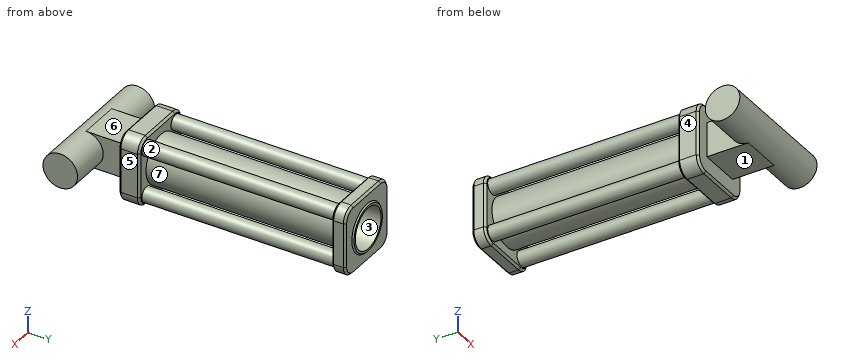
```python
from build123d import *

# Parameters (mm, degrees)
SKETCH1_R                = 175
SKETCH1_R_2              = 150
BOSS_EXTRUDE1_DEPTH      = 1500
SKETCH2_W                = 500
SKETCH2_H                = 500
BOSS_EXTRUDE2_DEPTH      = 150
BOSS_EXTRUDE3_DEPTH      = 150
BOSS_EXTRUDE3_DEPTH_BACK = 150
BOSS_EXTRUDE4_DEPTH      = 450
BOSS_EXTRUDE4_DEPTH_BACK = 450
SKETCH4_R                = 125
CHAMFER2_SIZE            = 10
SKETCH5_W                = 500
SKETCH5_H                = 500
SKETCH5_R                = 154.887495166
BOSS_EXTRUDE5_DEPTH      = 100
BOSS_EXTRUDE6_REACH      = 1587.875
SKETCH6_R                = 54.226637303
CIRPATTERN1_COUNT        = 4
FILLET1_R                = 90
CHAMFER3_SIZE            = 15


with BuildPart() as part:
    # Sketch1 → Boss-Extrude1 (new body)
    with BuildSketch(Plane(origin=(0, 0, 0), x_dir=(1, 0, 0), z_dir=(0, 1, 0))):
        with Locations(Location((0, 0, 0), (0, 0, 270))):
            Circle(SKETCH1_R)
        with Locations(Location((0, 0, 0), (0, 0, 270))):
            Circle(SKETCH1_R_2, mode=Mode.SUBTRACT)
    extrude(amount=BOSS_EXTRUDE1_DEPTH)

    # Sketch2 → Boss-Extrude2 (add)
    with BuildSketch(Plane.XZ):
        Rectangle(SKETCH2_W, SKETCH2_H)
    extrude(amount=BOSS_EXTRUDE2_DEPTH)

    # Sketch3 → Boss-Extrude3 (add, two sides: drawn at the far end of the back side and taken through both)
    with BuildSketch(Plane(origin=(0, 0, 0), x_dir=(0, 0, -1), z_dir=(1, 0, 0)).offset(-BOSS_EXTRUDE3_DEPTH_BACK)):
        with BuildLine():
            Line((125, -150), (125, -450))
            ThreePointArc((125, -450), (0, -575), (-125, -450))
            Line((-125, -450), (-125, -150))
            Line((-125, -150), (125, -150))
        make_face()
    extrude(amount=BOSS_EXTRUDE3_DEPTH + BOSS_EXTRUDE3_DEPTH_BACK)

    # Sketch4 → Boss-Extrude4 (add, two sides: drawn at the far end of the back side and taken through both)
    with BuildSketch(Plane(origin=(0, 0, 0), x_dir=(0, 0, -1), z_dir=(1, 0, 0)).offset(-BOSS_EXTRUDE4_DEPTH_BACK)):
        with Locations((0, -450)):
            Circle(SKETCH4_R)
    extrude(amount=BOSS_EXTRUDE4_DEPTH + BOSS_EXTRUDE4_DEPTH_BACK)

    # Chamfer2
    chamfer2_edges = [part.edges().sort_by_distance(p)[0] for p in [
        (0, 1500, -175),
    ]]
    chamfer(chamfer2_edges, length=CHAMFER2_SIZE)

    # Sketch5 → Boss-Extrude5 (add)
    with BuildSketch(Plane(origin=(0, 1490, 0), x_dir=(1, 0, 0), z_dir=(0, 1, 0))):
        Rectangle(SKETCH5_W, SKETCH5_H)
        Circle(SKETCH5_R, mode=Mode.SUBTRACT)
    extrude(amount=-BOSS_EXTRUDE5_DEPTH)

    # Sketch6 → Boss-Extrude6 (add, up to next)
    with BuildSketch(Plane(origin=(0, 0, 0), x_dir=(1, 0, 0), z_dir=(0, 1, 0)), mode=Mode.PRIVATE) as boss_extrude6_sk1:
        with Locations(Location((-170.275340777, 170.275340777, 0), (0, 0, 90))):
            Circle(SKETCH6_R)
    boss_extrude6_tool1 = extrude(boss_extrude6_sk1.sketch, amount=BOSS_EXTRUDE6_REACH, mode=Mode.PRIVATE) - part.part
    boss_extrude6 = boss_extrude6_tool1.solids().sort_by_distance((-170.275341, 0, -170.275341))[0]
    add(boss_extrude6)

    # CirPattern1: Boss-Extrude6 ×4 about axis
    cirpattern1_axis = Axis((0, 0, 0), (0, 1, 0))
    for i in range(1, CIRPATTERN1_COUNT):
        add(boss_extrude6.rotate(cirpattern1_axis, i * 360 / CIRPATTERN1_COUNT))

    # Fillet1
    fillet1_edges = [part.edges().sort_by_distance(p)[0] for p in [
        (250, -75, -250),
        (250, -75, 250),
        (-250, -75, 250),
        (-250, -75, -250),
        (250, 1440, -250),
        (250, 1440, 250),
        (-250, 1440, 250),
        (-250, 1440, -250),
    ]]
    fillet(fillet1_edges, radius=FILLET1_R)

    # Chamfer3
    chamfer3_edges = [part.edges().sort_by_distance(p)[0] for p in [
        (250, -150, 0),
        (0, 0, -250),
        (-250, 0, 0),
        (0, 0, 250),
        (-223.639610307, 0, -223.639610307),
        (-223.639610307, 0, 223.639610307),
        (223.639610307, 0, 223.639610307),
        (223.639610307, 0, -223.639610307),
        (0, -150, -250),
        (0, -150, 250),
        (-250, -150, 0),
        (-223.639610307, -150, -223.639610307),
        (-223.639610307, -150, 223.639610307),
        (223.639610307, -150, 223.639610307),
        (223.639610307, -150, -223.639610307),
        (0, 1490, -250),
        (0, 1390, -250),
        (250, 1490, 0),
        (-250, 1490, 0),
        (0, 1490, 250),
        (223.639610307, 1490, -223.639610307),
        (223.639610307, 1490, 223.639610307),
        (-223.639610307, 1490, 223.639610307),
        (-223.639610307, 1490, -223.639610307),
        (-250, 1390, 0),
        (250, 1390, 0),
        (0, 1390, 250),
        (223.639610307, 1390, -223.639610307),
        (223.639610307, 1390, 223.639610307),
        (-223.639610307, 1390, 223.639610307),
        (-223.639610307, 1390, -223.639610307),
        (250, 0, 0),
    ]]
    chamfer(chamfer3_edges, length=CHAMFER3_SIZE)


solid = part.part
```
Read the model definition and answer for the solid it produces. Units are mm, in the model's axes. Face numbers are marked on the shaded views. A direction names the side the tool comes from. Coordinates: 2 decimals unless noted, no trailing zeros. Order: outer loops, then holes, each group sorted by start corner. A loop starts at its lowest first (then second) coordinate and runs counter-clockwise, first axis right, second up. Notation, with made-up numbers: (33.5, -6.75) - (75.5, -6.75) arc R19 cw to (75.5, 2.25) - close; hole circle Ø3 at (-11, 67.5). An arc over 180 degrees is marked (long way). Answer as a JSON object with one key per item and string values. Group by question number.
Item 1: A tool of negligible diameter and unlimited length cuts with its end or side. For the marked faces 1, 2, 3 and 4, from which of +Z, -Z, +X, -X, +Y, -Y can it reach the whole face along a straight path? Write none if from no direction.
Item 2: Consider probe 1 along Z at (x, y) = (9, 765.5); probe 2 along X at (y, z) = (392, 0); probe 3 along Y at (x, z) = (-241, -52). Determine where each line is inside the solid, lowest interval first. Write a range as from..to.
Item 3: Flat-ended cylindrical pins translate along their axes: P1, Ø12, axis at x = 0, z = -30.5, coming from the +Y side; P2, Ø12, axis at x = -171.5, y = 787.5, coming from the +Z side; P3, Ø12, axis at y = -276.5, z = -68, coming from the +X side. Find the tip coordinate at first contact, or state that the pin passes through.
Item 4: Section C-C (x = -348) is taken. Give the vertices of the cut face in (y, z).
Item 5: The mould has two halves that part along Z. Classify the marked faces 5, 6 and 7: +Z half, -Z half, draft (parallel to the pull), parting line (faces both ways), or undercut.
Item 6: Section A-A (y = 298.5) is taken. Give the vertices of the cut face in (x, z), plus the area to 3 significant figures.
Results are:
{
 "1": {"face 1": "-Z, +X, -X, -Y", "face 2": "none", "face 3": "+Y", "face 4": "+Z, -Z, -X, +Y"},
 "2": {"probe 1": "z = -174.77..-149.73, 149.73..174.77", "probe 2": "x = -175..-150, 150..175", "probe 3": "y = -563.67..-336.33, -144..-6, 1396..1484"},
 "3": {"P1": "stops at y = 0", "P2": "stops at z = 224.5", "P3": "stops at x = 150"},
 "4": {"outline": "circle Ø250 at (-450, 0)"},
 "5": {"face 5": "draft", "face 6": "+Z half", "face 7": "undercut"},
 "6": {"outline": "circle Ø108.45 at (-170.28, -170.28); circle Ø108.45 at (-170.28, 170.28); circle Ø350 at (0, 0); circle Ø108.45 at (170.28, -170.28); circle Ø108.45 at (170.28, 170.28); hole circle Ø300 at (0, 0)", "area": "62,500 mm^2"}
}
